from build123d import *

# Parameters (mm, degrees)
BASE_PROFILE_SKETCH_R             = 7
BASE_BODY_DEPTH                   = 55
RECESS_PROFILE_SKETCH_W           = 28
RECESS_PROFILE_SKETCH_H           = 40.468356276
RECESS_CUT_78_DEPTH               = 39
EYELET_LUG_SKETCH_R               = 22.5
EYELET_LUG_SKETCH_R_2             = 10
EYELET_LUG_20_DEPTH               = 20
EYELET_WEB_12_DEPTH               = 12
COUNTERBORED_HOLES_12_D           = 12
COUNTERBORED_HOLES_12_CBORE_D     = 24
COUNTERBORED_HOLES_12_CBORE_DEPTH = 6


with BuildPart() as part:
    # Base Profile Sketch → Base Body (new, symmetric)
    with BuildSketch(Plane(origin=(0, 0, 0), x_dir=(0, 0, -1), z_dir=(1, 0, 0))):
        with BuildLine():
            Line((40, 0), (20, 0))
            Line((20, 0), (20, 15))
            Line((20, 15), (0, 15))
            Line((0, 15), (0, 0))
            Line((0, 0), (-56, 0))
            ThreePointArc((-56, 0), (-69.379366808, 9.877798669), (-63.878920524, 25.572493741))
            Line((-63.878920524, 25.572493741), (-28, 50))
            Line((-28, 50), (-16, 50))
            Line((-16, 50), (-16, 35))
            Line((-16, 35), (40, 35))
            Line((40, 35), (40, 0))
        make_face()
        with Locations((-56, 14)):
            Circle(BASE_PROFILE_SKETCH_R, mode=Mode.SUBTRACT)
    extrude(amount=BASE_BODY_DEPTH, both=True)

    # Recess Profile Sketch → Recess Cut 78 (cut, symmetric)
    with BuildSketch(Plane(origin=(0, 0, 0), x_dir=(0, 0, -1), z_dir=(1, 0, 0))):
        with Locations((-56, 20.234178138)):
            Rectangle(RECESS_PROFILE_SKETCH_W, RECESS_PROFILE_SKETCH_H)
    extrude(amount=RECESS_CUT_78_DEPTH, both=True, mode=Mode.SUBTRACT)



with BuildPart() as body_2:
    # Eyelet Lug Sketch → Eyelet Lug 20 (new body)
    with BuildSketch(Plane(origin=(0, 0, 16), x_dir=(-1, 0, 0), z_dir=(0, 0, -1))):
        with Locations((0, 83)):
            Circle(EYELET_LUG_SKETCH_R)
        with Locations((0, 83)):
            Circle(EYELET_LUG_SKETCH_R_2, mode=Mode.SUBTRACT)
    extrude(amount=-EYELET_LUG_20_DEPTH)


with BuildPart() as part_1:
    add(part.part)

    add(body_2.part)  # Eyelet Web 12 merges body 2
    # Sketch4_3 → Eyelet Web 12 (add)
    with BuildSketch(Plane(origin=(0, 0, 16), x_dir=(-1, 0, 0), z_dir=(0, 0, -1))):
        with BuildLine():
            Line((-35, 50), (0, 50))
            Line((0, 50), (0, 60.5))
            ThreePointArc((0, 60.5), (-18.294452315, 69.901793463), (-21.299956881, 90.249954267))
            Line((-21.299956881, 90.249954267), (-35, 50))
        make_face()
        with BuildLine():
            Line((0, 60.5), (0, 50))
            Line((0, 50), (35, 50))
            Line((35, 50), (21.299956881, 90.249954267))
            ThreePointArc((21.299956881, 90.249954267), (22.197961954, 86.674300626), (22.5, 83))
            ThreePointArc((22.5, 83), (15.909902577, 67.090097423), (0, 60.5))
        make_face()
    extrude(amount=-EYELET_WEB_12_DEPTH)

    # Counterbored Holes _12 (through all)
    with Locations(Plane(origin=(0, 35, 0), x_dir=(1, 0, 0), z_dir=(0, 1, 0))):
        with Locations((35, 14), (0, 14), (-35, 14)):
            CounterBoreHole(COUNTERBORED_HOLES_12_D / 2, COUNTERBORED_HOLES_12_CBORE_D / 2, COUNTERBORED_HOLES_12_CBORE_DEPTH)


solid = part_1.part
The listing builds one solid part. Answer for the finished solid, in the listing's coordinates (mm). A direction names the side the tool comes from. Give positions to 0.01 mm unless a question says otherwise; leave off trailing zeros. Order: outer loops, then holes, each group sorted by start corner. A loop starts at its lowest first (then second) coordinate and runs counter-clockwise, first axis right, second up. Notation, with made-up numbers: (-39, 10.5) -> (-6, 10.5) arc R14 ccw to (-6, 25.5) -> close; hole circle Ø3 at (80.25, 59). An arc over 180 degrees is marked (long way). Put each result on its own line as item: value.
Item 1: A cutting plane is placed at B-B on x = -3.5. Give the vertices of the cut face in (y, z).
Established:
outline: (0, -40) -> (35, -40) -> (35, -25.48) -> (29, -25.48) -> (29, -18.87) -> (15, -18.87) -> (15, -20) -> (0, -20) -> close; (0, 0) -> (15, 0) -> (15, -9.13) -> (29, -9.13) -> (29, -2.52) -> (35, -2.52) -> (35, 16) -> (73.63, 16) -> (73.63, 36) -> (60.77, 36) -> (60.77, 28) -> (50, 28) -> (40.47, 42) -> (0, 42) -> close; (92.37, 16) -> (105.23, 16) -> (105.23, 36) -> (92.37, 36) -> close
Item 2: Given P1, Ø5, axis at x = -42.5, y = 20.5, coming from the +Z side; P2, Ø15.5, axis at x = 0, z = -14, coming from the +Y side; P3, Ø8, axis at x = -13, y = 72.5, coming from the -Z side; P4, Ø19, axis at x = -35, z = -14, coming from the -Y side, each flat-ended and moving along its own axis, determine where each tip first touches the part or whether it passes through.
Established:
P1: stops at z = 69.42
P2: stops at y = 29
P3: stops at z = 16
P4: stops at y = 0
Item 3: A cutting plane is placed at C-C on y = 83. Give the vertices of the cut face in (x, z), plus the area to 3 significant figures.
Established:
outline: (-23.77, 16) -> (-10, 16) -> (-10, 36) -> (-22.5, 36) -> (-22.5, 28) -> (-23.77, 28) -> close; (10, 16) -> (23.77, 16) -> (23.77, 28) -> (22.5, 28) -> (22.5, 36) -> (10, 36) -> close
area: 530 mm^2
Item 4: A cutting plane is placed at A-A on z = -14. Give the vertices of the cut face in (x, y), plus the area to 3 significant figures.
Established:
outline: (-55, 15) -> (-41, 15) -> (-41, 29) -> (-47, 29) -> (-47, 35) -> (-55, 35) -> close; (-29, 15) -> (-6, 15) -> (-6, 29) -> (-12, 29) -> (-12, 35) -> (-23, 35) -> (-23, 29) -> (-29, 29) -> close; (6, 15) -> (29, 15) -> (29, 29) -> (23, 29) -> (23, 35) -> (12, 35) -> (12, 29) -> (6, 29) -> close; (41, 15) -> (55, 15) -> (55, 35) -> (47, 35) -> (47, 29) -> (41, 29) -> close
area: 1,260 mm^2
Item 5: For a pull along X with two mould halves and no side action, classify faces 4 (the face through (-55, 20, 14)), 5 (the face through (39, 21, 53)), 6 (the face through (47.112, 9.64, 69.304)) as released by +X, released by -X, zero draft, split by the parting line, or undercut.
Established:
face 4: released by -X
face 5: undercut
face 6: zero draft
Item 6: A cutting plane is placed at D-D on z = 21. Give the vertices of the cut face in (x, y), plus the area to 3 significant figures.
Established:
outline: (-55, 0) -> (55, 0) -> (55, 50) -> (35, 50) -> (21.3, 90.25) arc R22.5 ccw to (-21.3, 90.25) -> (-35, 50) -> (-55, 50) -> close; hole circle Ø20 at (0, 83)
area: 7,930 mm^2
Item 7: For faces 1 (the face through (-45, 50, 22)), 2 (the face through (-1.56, 32.04, -25.9)), 3 (the face through (0.8, 15, -7.9)), determine the directions among +Z, -Z, +X, -X, +Y, -Y from which every point of the face is accessible in a straight line to the end or side of a thin tool.
Established:
face 1: +Z, -Z, -X, +Y
face 2: +Y
face 3: +X, -X, -Y
Item 8: Straight lines are drawn through the part: line 1 (X direction, y = 7, z = 66); line 2 (Z direction, x = 41.5, y = 12); line 3 (Y direction, x = 28, z = -3). For each, find the intervals that lie inside material, in ascending order.
Established:
line 1: x = -55 to -39, 39 to 55
line 2: z = -40 to -20, 0 to 49.29, 62.71 to 69.86
line 3: y = 15 to 35
